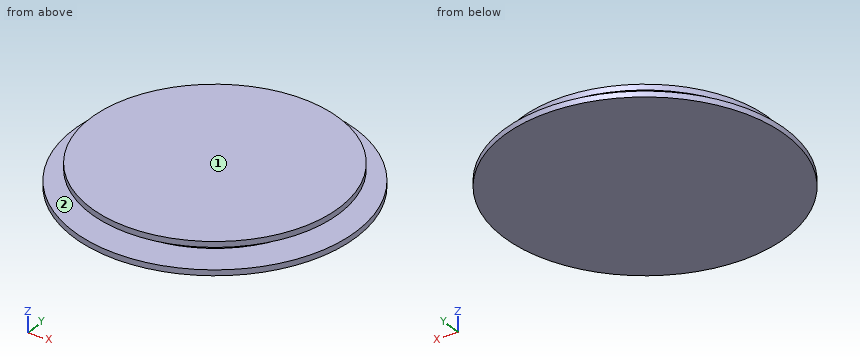
from build123d import *

# Parameters (mm, degrees)
SKETCH_3_R           = 25
BOSS_EXTRUDE_1_DEPTH = 1
SKETCH_4_R           = 19
BOSS_EXTRUDE_2_DEPTH = 2
SKETCH_5_R           = 22
BOSS_EXTRUDE_3_DEPTH = 1


with BuildPart() as part:
    # Sketch 3 → Boss-Extrude 1 (new body)
    with BuildSketch(Plane.XY):
        Circle(SKETCH_3_R)
    extrude(amount=BOSS_EXTRUDE_1_DEPTH)

    # Sketch 4 → Boss-Extrude 2 (add)
    with BuildSketch(Plane.XY.offset(1)):
        Circle(SKETCH_4_R)
    extrude(amount=BOSS_EXTRUDE_2_DEPTH)

    # Sketch 5 → Boss-Extrude 3 (add)
    with BuildSketch(Plane.XY.offset(3)):
        Circle(SKETCH_5_R)
    extrude(amount=BOSS_EXTRUDE_3_DEPTH)


solid = part.part
Design review of the part built by this model. Coordinates are the model's own, in mm. Face numbers are marked on the shaded views. A direction names the side the tool comes from. Give positions to 0.01 mm unless a question says otherwise; leave off trailing zeros. Write each loop counter-clockwise with the first axis right and the second up, starting at its lowest first coordinate (ties: lowest second). Pieces come first, ordered by that corner, then holes. Notation, with made-up numbers: M 10,-14 L 65,-14 A23 cw 65,24 Z; hole C -1.75,85 d6. An arc over 180 degrees is marked long. Answer as a JSON object with one key per item and string values. Group by question number.
1) For line 1 along Z through (x, y) = (-3.5, -20); line 2 along Z through (x, y) = (20, 14); line 3 along Y through (x, z) = (-0.5, 3.65), list the stretches that pass through material, from the lowest coordinate up.
2) We need section A-A (y = 0). Give the boundary of the cut face in (x, z).
3) We need section C-C (z = 1.75). Give the boundary of the cut face in (x, y), and give its area (3 significant figures).
4) Tool access review of the marked faces 1 and 2: name each direction out of +Z, -Z, +X, -X, +Y, -Y from which nothing blocks a thin tool from reaching the whole face with its end or side.
5) Clearance check with flat-ended pins moving along their axes: pin 1 Ø1.5 at (y, z) = (11.5, 1.5) entering from -X; pin 2 Ø1.5 at (y, z) = (-15.5, 1) entering from +X; pin 3 Ø1 at (x, z) = (-14, 1) entering from +Y. State where each tip first meets the part, or that it passes through.
Answer key:
{
 "1": {"line 1": "z = 0 to 1, 3 to 4", "line 2": "z = 0 to 1", "line 3": "y = -21.99 to 21.99"},
 "2": {"outline": "M -25,0 L 25,0 L 25,1 L 19,1 L 19,3 L 22,3 L 22,4 L -22,4 L -22,3 L -19,3 L -19,1 L -25,1 Z"},
 "3": {"outline": "C 0,0 d38", "area": "1,130 mm²"},
 "4": {"face 1": "+Z, +X, -X, +Y, -Y", "face 2": "none"},
 "5": {"pin 1": "stops at x = -22.48", "pin 2": "stops at x = 20.19", "pin 3": "stops at y = 21.04"}
}
